from build123d import *

# Parameters (mm, degrees)
SKETCH1_W                  = 58
SKETCH1_H                  = 39.5
SKETCH1_R                  = 8.5
SKETCH1_R_2                = 3
BOSS_EXTRUDE1_DEPTH        = 6
M3_TAPPED_HOLE1_D          = 2.5
M4_TAPPED_HOLE1_AT_2_COUNT = 2
M4_TAPPED_HOLE1_AT_2_PITCH = 41
CHAMFER1_SIZE              = 1
CHAMFER2_SIZE              = 0.5


with BuildPart() as part:
    # Sketch1 → Boss-Extrude1 (new, symmetric)
    with BuildSketch(Plane.XY):
        Rectangle(SKETCH1_W, SKETCH1_H)
        with Locations((0, -5.25)):
            Circle(SKETCH1_R, mode=Mode.SUBTRACT)
        with Locations((-20.5, -8.75)):
            Circle(SKETCH1_R_2, mode=Mode.SUBTRACT)
        with Locations((20.5, -8.75)):
            Circle(SKETCH1_R_2, mode=Mode.SUBTRACT)
    extrude(amount=BOSS_EXTRUDE1_DEPTH, both=True)

    # M3 Tapped Hole1 (through all)
    with Locations(Plane.XY.offset(6)):
        with Locations((-14.5, 2.25), (14.5, -12.75)):
            Hole(M3_TAPPED_HOLE1_D / 2)

    # Sketch4 → M4 Tapped Hole1 (revolve, cut)
    with BuildSketch(Plane(origin=(-20.5, -19.75, 0), x_dir=(0, 0, -1), z_dir=(1, 0, 0))):
        Polygon((0, 0), (0, 11.091420021), (1.65, 10.1), (1.65, 0), align=None)
    m4_tapped_hole1 = revolve(axis=Axis((-20.5, -26.1, 0), (0, 1, 0)), mode=Mode.SUBTRACT)

    # M4 Tapped Hole1 at 2: M4 Tapped Hole1 ×2
    with Locations(*[(i * M4_TAPPED_HOLE1_AT_2_PITCH, 0, 0) for i in range(1, M4_TAPPED_HOLE1_AT_2_COUNT)]):
        add(m4_tapped_hole1, mode=Mode.SUBTRACT)

    # Mirror1: M4 Tapped Hole1 across plane
    add(m4_tapped_hole1.mirror(Plane.ZX), mode=Mode.SUBTRACT)

    # Mirror1 copy 1 sketch → Mirror1 copy 1 (revolve, cut)
    with BuildSketch(Plane(origin=(20.5, 19.75, 0), x_dir=(0, 0, -1), z_dir=(1, 0, 0))):
        Polygon((0, 0), (0, -11.091420021), (1.65, -10.1), (1.65, 0), align=None)
    revolve(axis=Axis((20.5, 26.1, 0), (0, 1, 0)), mode=Mode.SUBTRACT)

    # Chamfer1
    chamfer1_edges = [part.edges().sort_by_distance(p)[0] for p in [
        (29, -19.75, 0),
        (-29, -19.75, 0),
        (-29, 19.75, 0),
        (29, 19.75, 0),
    ]]
    chamfer(chamfer1_edges, length=CHAMFER1_SIZE)

    # Chamfer2
    chamfer2_edges = [part.edges().sort_by_distance(p)[0] for p in [
        (-8.5, -5.25, -6),
        (-8.5, -5.25, 6),
    ]]
    chamfer(chamfer2_edges, length=CHAMFER2_SIZE)


solid = part.part
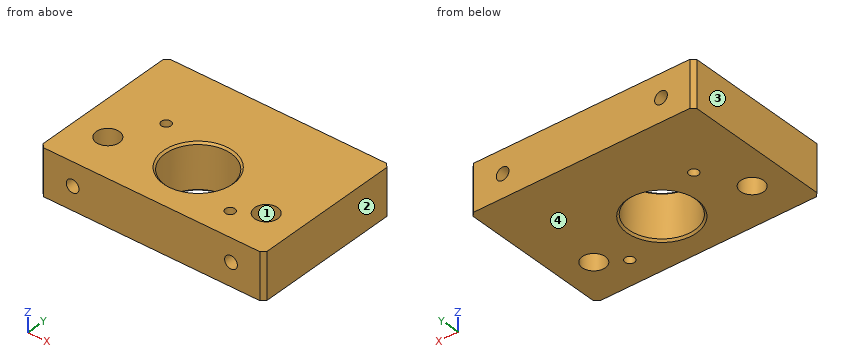
Model file for the job. Use its own axes, mm. Face numbers are marked on the shaded views. Coordinates: 2 decimals unless noted, no trailing zeros. Order: outer loops, then holes, each group sorted by start corner. A loop starts at its lowest first (then second) coordinate and runs counter-clockwise, first axis right, second up. Notation, with made-up numbers: (71.25, 49.25) -> (97.25, 49.25) arc R21 ccw to (97.25, 69.25) -> close; hole circle Ø6 at (-17, 27.5). An arc over 180 degrees is marked (long way). Return JSON: item names as keys, results as strings. Group by question number.
Item 1: Saw through at D-D on x = 0. Write the cut outline in (y, z).
Item 2: Saw through at C-C on y = 13.5. Write the cut outline in (x, z).
Item 3: Wall check: line 1 along X through (y, z) = (13, 0); line 2 along Y through (x, z) = (14.5, -1.5); line 3 along X through (y, z) = (-8, 1). Give the ranges that are in metal, low to high. Write a range as [from, to].
Item 4: Flat gauge pins, fed straight in: P1, Ø2, axis at x = -20.5, z = 0, coming from the +Y side; P2, Ø3, axis at x = 20.5, z = 0, coming from the -Y side; P3, Ø2, axis at x = -14.5, y = 2.25, coming from the +Z side. Where does each tip first touch, or does it go through?
Item 5: Saw through at A-A on x = -14.5. Write the cut outline in (y, z).
Item 6: Saw through at B-B on z = 4.75. Write the cut outline in (x, y).
Item 7: Pull direction X, two halves, no side cores. Call the marked faces 1, 2, 3 and 4: pulls with the +X half, pulls with the -X half, needs draft (parallel to the pull), parting line crosses it, or undercut.
Values found:
{
 "1": {"outline": "(-19.75, -6) -> (-14.25, -6) -> (-13.75, -5.5) -> (-13.75, 5.5) -> (-14.25, 6) -> (-19.75, 6) -> close; (3.25, -5.5) -> (3.75, -6) -> (19.75, -6) -> (19.75, 6) -> (3.75, 6) -> (3.25, 5.5) -> close"},
 "2": {"outline": "(-29, -6) -> (29, -6) -> (29, 6) -> (-29, 6) -> close; hole circle Ø3.3 at (-20.5, 0); hole circle Ø3.3 at (20.5, 0)"},
 "3": {"line 1": "x = [-29, -22.15], [-18.85, 18.85], [22.15, 29]", "line 2": "y = [-19.75, -14], [-11.5, 19.75]", "line 3": "x = [-29, -23.4], [-17.6, -8.04], [8.04, 17.6], [23.4, 29]"},
 "4": {"P1": "stops at y = 9.26", "P2": "stops at y = -6.15", "P3": "passes through"},
 "5": {"outline": "(-19.75, -6) -> (1, -6) -> (1, 6) -> (-19.75, 6) -> close; (3.5, -6) -> (19.75, -6) -> (19.75, 6) -> (3.5, 6) -> close"},
 "6": {"outline": "(-29, -18.75) -> (-28, -19.75) -> (28, -19.75) -> (29, -18.75) -> (29, 18.75) -> (28, 19.75) -> (-28, 19.75) -> (-29, 18.75) -> close; hole circle Ø6 at (-20.5, -8.75); hole circle Ø2.5 at (-14.5, 2.25); hole circle Ø17 at (0, -5.25); hole circle Ø2.5 at (14.5, -12.75); hole circle Ø6 at (20.5, -8.75)"},
 "7": {"face 1": "undercut", "face 2": "pulls with the +X half", "face 3": "pulls with the -X half", "face 4": "needs draft"}
}
